```python
from build123d import *

# Parameters (mm, degrees)
BASE_PLATE_SKETCH_W          = 80
BASE_PLATE_SKETCH_H          = 80
BASE_PLATE_80X80X20_DEPTH    = 20
BOTTOM_SLOT_SKETCH_W         = 25
BOTTOM_SLOT_SKETCH_H         = 5
BOTTOM_SLOT_SKETCH_W_2       = 35
BOTTOM_SLOT_DEPTH            = 80
RAISED_BLOCK_SKETCH_W        = 80
RAISED_BLOCK_SKETCH_H        = 60
RAISED_BLOCK_DEPTH           = 20
BLOCK_STEP_CUT_1_SKETCH_W    = 15
BLOCK_STEP_CUT_1_SKETCH_H    = 10
BLOCK_STEP_CUT_1_DEPTH       = 20
BLOCK_STEP_CUT_2_DEPTH       = 20
BLOCK_ANGLE_CUT_30DEG_REACH  = 102.233
COUNTERBORE_25_SKETCH_R      = 10
COUNTERBORE_25X5_DEPTH       = 5
HOLE_10_SKETCH_R             = 5
HOLE_10X10_DEPTH             = 10
AUXILIARY_BODY_EXTRUDE_DEPTH = 50
AUXILIARY_BODY_FILLET_R20_R  = 20


with BuildPart() as part:
    # Base Plate Sketch → Base Plate 80x80x20 (new body)
    with BuildSketch(Plane(origin=(0, 0, 0), x_dir=(1, 0, 0), z_dir=(0, 1, 0))):
        with Locations((5.239833721, 5.239833721)):
            Rectangle(BASE_PLATE_SKETCH_W, BASE_PLATE_SKETCH_H)
    extrude(amount=BASE_PLATE_80X80X20_DEPTH)

    # Bottom Slot Sketch → Bottom Slot (cut)
    with BuildSketch(Plane(origin=(45.239833721, 0, 0), x_dir=(0, 0, -1), z_dir=(1, 0, 0))):
        with Locations((-22.260166279, 2.5)):
            Rectangle(BOTTOM_SLOT_SKETCH_W, BOTTOM_SLOT_SKETCH_H)
        with Locations((27.739833721, 2.5)):
            Rectangle(BOTTOM_SLOT_SKETCH_W_2, BOTTOM_SLOT_SKETCH_H)
    extrude(amount=-BOTTOM_SLOT_DEPTH, mode=Mode.SUBTRACT)

    # Raised Block Sketch → Raised Block (add)
    with BuildSketch(Plane(origin=(0, 20, 0), x_dir=(1, 0, 0), z_dir=(0, 1, 0))):
        with Locations((5.239833721, 15.239833721)):
            Rectangle(RAISED_BLOCK_SKETCH_W, RAISED_BLOCK_SKETCH_H)
    extrude(amount=RAISED_BLOCK_DEPTH)

    # Block Step Cut 1 Sketch → Block Step Cut 1 (cut)
    with BuildSketch(Plane(origin=(0, 40, 0), x_dir=(1, 0, 0), z_dir=(0, 1, 0))):
        with Locations((37.739833721, 40.239833721)):
            Rectangle(BLOCK_STEP_CUT_1_SKETCH_W, BLOCK_STEP_CUT_1_SKETCH_H)
    extrude(amount=-BLOCK_STEP_CUT_1_DEPTH, mode=Mode.SUBTRACT)

    # Block Step Cut 2 Sketch → Block Step Cut 2 (cut)
    with BuildSketch(Plane(origin=(0, 40, 0), x_dir=(1, 0, 0), z_dir=(0, 1, 0))):
        Polygon((30.239833721, 35.239833721), (-19.760166279, -14.760166279), (45.239833721, -14.760166279), (45.239833721, 35.239833721), align=None)
    extrude(amount=-BLOCK_STEP_CUT_2_DEPTH, mode=Mode.SUBTRACT)

    # Block Angle Cut 30deg Sketch → Block Angle Cut 30deg (cut, up to next)
    with BuildSketch(Plane(origin=(0, 0, -45.239833721), x_dir=(-1, 0, 0), z_dir=(0, 0, -1)), mode=Mode.PRIVATE) as block_angle_cut_30deg_sk1:
        Polygon((34.760166279, 40), (7.167951709, 40), (34.760166279, 24.06962749), align=None)
    block_angle_cut_30deg_tool1 = extrude(block_angle_cut_30deg_sk1.sketch, amount=-BLOCK_ANGLE_CUT_30DEG_REACH, mode=Mode.PRIVATE) & part.part
    add(block_angle_cut_30deg_tool1.solids().sort_by_distance((-25.562761, 34.689876, -45.239834))[0], mode=Mode.SUBTRACT)

    # Counterbore Ø25 Sketch → Counterbore Ø25x5 (cut)
    with BuildSketch(Plane(origin=(0, 20, 0), x_dir=(1, 0, 0), z_dir=(0, 1, 0))):
        with Locations(Location((20.239833721, 0.239833721, 0), (0, 0, 270))):
            Circle(COUNTERBORE_25_SKETCH_R)
    extrude(amount=-COUNTERBORE_25X5_DEPTH, mode=Mode.SUBTRACT)

    # Hole Ø10 Sketch → Hole Ø10x10 (cut)
    with BuildSketch(Plane(origin=(0, 15, 0), x_dir=(1, 0, 0), z_dir=(0, 1, 0))):
        with Locations(Location((20.239833721, 0.239833721, 0), (0, 0, 270))):
            Circle(HOLE_10_SKETCH_R)
    extrude(amount=-HOLE_10X10_DEPTH, mode=Mode.SUBTRACT)


with BuildPart() as body_2:
    # Auxiliary Body Profile Sketch → Auxiliary Body Extrude (new, symmetric)
    with BuildSketch(Plane.XY):
        Polygon((417.503137043, -16.766117227), (417.503137043, -472.594475264), (451.565036325, -472.594475264), (451.565036325, -269.453576574), (494.657405519, -220.272068254), (589.816274586, -472.594475264), (625.881815002, -472.594475264), (519.87061451, -191.49612321), (672.967381657, -16.766117227), (635.900020673, -16.766117227), (451.565036325, -227.148436321), (451.565036325, -16.766117227), align=None)
    extrude(amount=AUXILIARY_BODY_EXTRUDE_DEPTH, both=True)

    # Auxiliary Body Fillet R20
    auxiliary_body_fillet_r20_edges = [body_2.edges().sort_by_distance(p)[0] for p in [
        (451.565036325, -227.148436321, 0),
        (519.87061451, -191.49612321, 0),
        (451.565036325, -269.453576574, 0),
    ]]
    fillet(auxiliary_body_fillet_r20_edges, radius=AUXILIARY_BODY_FILLET_R20_R)


solid = part.part
```
Geometry check sheet. Reference: the model listing, model coordinates, mm. A direction names the side the tool comes from. Coordinates: 2 decimals unless noted, no trailing zeros. Order: outer loops, then holes, each group sorted by start corner. A loop starts at its lowest first (then second) coordinate and runs counter-clockwise, first axis right, second up. Notation, with made-up numbers: (82, -2) - (98, -2) arc R14 ccw to (98, 2) - close; hole circle Ø1 at (33, 43.5). An arc over 180 degrees is marked (long way). Answer in a Markdown table with one row per item. Add a question column.
1. Gauge pin test, flat ends, axial feed: pin 1 Ø3 at (y, z) = (26.5, -38.5) entering from +X; pin 2 Ø6 at (x, z) = (23, 2.5) entering from +Y; pin 3 Ø23 at (x, z) = (20.24, -0.24) entering from +Y. Record the tip position at first contact, or that the pin passes through.
2. Material ranges on L1, parallel to Y at x = 30.5, z = 7; L2, parallel to Y at x = 14, z = 26; L3, parallel to Z at x = 22.5, y = 16.5, recorded low to high. Write a range as [from, to].
3. Section check C-C (y = 16). Enter the section's corners in (x, z).
4. Section check A-A (x = 8). Enter the section's corners in (y, z).
5. Section check D-D (x = 34). Enter the section's corners in (y, z), plus the area to 3 significant figures.
6. Draft check along Z on faces 4 (the face through (20, 5, 0)), 5 (the face through (6, 2, 9.76)), 6 (the face through (7, 40, -27)). Enter one of: +Z half, -Z half, draft (parallel to the pull), parting line (faces both ways), or undercut.
7. Access from +Z, -Z, +X, -X, +Y, -Y to the whole of each face (thin tool, end or side, straight path). Record for faces 1 (the face through (6, 5, 22)), 2 (the face through (-26, 25, 14.76)), 3 (the face through (6, 5, -27)).
8. Section check B-B (z = -19.5). Enter the section's corners in (x, y), plus the area to 3 significant figures.
Data:
| question | item | result |
|---|---|---|
| 1 | pin 1 | stops at x = 30.24 |
| 1 | pin 2 | stops at y = 15 |
| 1 | pin 3 | stops at y = 20 |
| 2 | L1 | y = [0, 20] |
| 2 | L2 | y = [5, 20] |
| 2 | L3 | z = [-45.24, -9.98], [9.5, 34.76] |
| 3 | outline | (-34.76, -45.24) - (45.24, -45.24) - (45.24, 34.76) - (-34.76, 34.76) - close; hole circle Ø20 at (20.24, -0.24) |
| 4 | outline | (0, -10.24) - (5, -10.24) - (5, -45.24) - (40, -45.24) - (40, -13) - (20, -13) - (20, 34.76) - (5, 34.76) - (5, 9.76) - (0, 9.76) - close |
| 5 | outline | (0, -10.24) - (5, -10.24) - (5, -45.24) - (20, -45.24) - (20, 34.76) - (5, 34.76) - (5, 9.76) - (0, 9.76) - close |
| 5 | area | 1,300 mm² |
| 6 | face 4 | undercut |
| 6 | face 5 | +Z half |
| 6 | face 6 | draft |
| 7 | face 1 | +Z, +X, -X, -Y |
| 7 | face 2 | +Z, +X, -X, +Y |
| 7 | face 3 | -Z, +X, -X, -Y |
| 8 | outline | (-34.76, 5) - (45.24, 5) - (45.24, 20) - (14.5, 20) - (14.5, 40) - (-7.17, 40) - (-34.76, 24.07) - close |
| 8 | area | 1,970 mm² |
